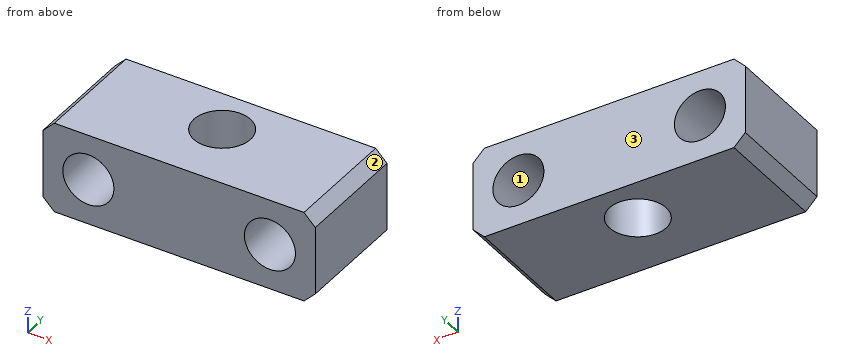
from build123d import *

# Parameters (mm, degrees)
SKETCH1_W                  = 24
SKETCH1_H                  = 10
BOSS_EXTRUDE1_DEPTH        = 4
F_4_5_4_5_DIAMETER_HOLE1_D = 4.5
CHAMFER1_SIZE              = 1
F_5_0_5_DIAMETER_HOLE1_D   = 5


with BuildPart() as part:
    # Sketch1 → Boss-Extrude1 (new, symmetric)
    with BuildSketch(Plane.XY):
        Rectangle(SKETCH1_W, SKETCH1_H)
    extrude(amount=BOSS_EXTRUDE1_DEPTH, both=True)

    # Ø4.5 (4.5) Diameter Hole1 (through all)
    with Locations(Plane(origin=(0, 5, 0), x_dir=(1, 0, 0), z_dir=(0, 1, 0))):
        with Locations((-8, 0), (8, 0)):
            Hole(F_4_5_4_5_DIAMETER_HOLE1_D / 2)

    # Chamfer1
    chamfer1_edges = [part.edges().sort_by_distance(p)[0] for p in [
        (-12, 0, 4),
        (12, 0, 4),
        (-12, 0, -4),
        (12, 0, -4),
    ]]
    chamfer(chamfer1_edges, length=CHAMFER1_SIZE)

    # Ø5.0 (5) Diameter Hole1 (through all)
    with Locations(Plane.XY.offset(4)):
        with Locations((0, 1)):
            Hole(F_5_0_5_DIAMETER_HOLE1_D / 2)


solid = part.part
Part model, mm, in its own coordinate system. Face numbers are marked on the shaded views. Give positions to 0.01 mm unless a question says otherwise; leave off trailing zeros. Order: outer loops, then holes, each group sorted by start corner. A loop starts at its lowest first (then second) coordinate and runs counter-clockwise, first axis right, second up. Notation, with made-up numbers: (18.5, 10) - (43.5, 10) arc R31 cw to (43.5, 45) - close; hole circle Ø9 at (-16.5, 54.5). An arc over 180 degrees is marked (long way). One line per question, with ' | ' between items.
1. Band-saw the part on B-B on z = 0. List the corners of the cut face in (x, y).
Filled in:
outline: (-12, -5) - (-10.25, -5) - (-10.25, 5) - (-12, 5) - close; (-5.75, -5) - (5.75, -5) - (5.75, 5) - (-5.75, 5) - close; (10.25, -5) - (12, -5) - (12, 5) - (10.25, 5) - close; hole circle Ø5 at (0, 1)
2. Pull direction Z, two halves, no side cores. Call the marked faces 1, 2 and 3: +Z half, -Z half, draft (parallel to the pull), parting line (faces both ways), or undercut.
Filled in:
face 1: undercut | face 2: +Z half | face 3: draft
3. Band-saw the part on D-D on y = -3. List the corners of the cut face in (x, z), then the cut area to 3 significant figures.
Filled in:
outline: (-12, -3) - (-11, -4) - (11, -4) - (12, -3) - (12, 3) - (11, 4) - (-11, 4) - (-12, 3) - close; hole circle Ø4.5 at (-8, 0); hole circle Ø4.5 at (8, 0) | area: 158 mm²
4. Band-saw the part on C-C on x = 0. List the corners of the cut face in (y, z).
Filled in:
outline: (-5, -4) - (-1.5, -4) - (-1.5, 4) - (-5, 4) - close; (3.5, -4) - (5, -4) - (5, 4) - (3.5, 4) - close
5. Drill centre lines: probe 1 along Z at (x, y) = (-8, -2); probe 2 along X at (y, z) = (-4.25, -0.75); probe 3 along X at (y, z) = (-2.75, 1.5). Where is each one in solid material? Low to high.
Filled in:
probe 1: -4 to -2.25, 2.25 to 4 | probe 2: -12 to -10.12, -5.88 to 5.88, 10.12 to 12 | probe 3: -12 to -9.68, -6.32 to 6.32, 9.68 to 12
6. Band-saw the part on A-A on y = 1. List the corners of the cut face in (x, z).
Filled in:
outline: (-12, -3) - (-11, -4) - (-2.5, -4) - (-2.5, 4) - (-11, 4) - (-12, 3) - close; (2.5, -4) - (11, -4) - (12, -3) - (12, 3) - (11, 4) - (2.5, 4) - close; hole circle Ø4.5 at (-8, 0); hole circle Ø4.5 at (8, 0)
